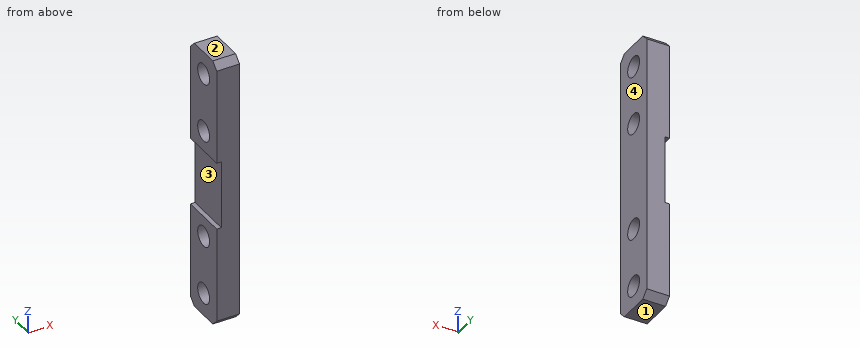
from build123d import *

# Parameters (mm, degrees)
SKETCH_1_W            = 120
SKETCH_1_H            = 20
EXTRUDE_1_DEPTH       = 10
HOLE_WIZARD_9_0_9_1_D = 9
HOLE_WIZARD_9_0_9_2_D = 9
SKETCH_6_W            = 30
SKETCH_6_H            = 20
CUT_EXTRUDE_1_DEPTH   = 2
CHAMFER_1_SIZE        = 3


with BuildPart() as part:
    # 草图1 → 凸台-拉伸1 (new body)
    with BuildSketch(Plane(origin=(0, 0, 0), x_dir=(0, 0, -1), z_dir=(1, 0, 0))):
        Rectangle(SKETCH_1_W, SKETCH_1_H)
    extrude(amount=EXTRUDE_1_DEPTH)

    # Ø9.0 (9) 直径孔1 (through all)
    with Locations(Plane(origin=(10, 0, 0), x_dir=(0, 0, -1), z_dir=(1, 0, 0))):
        with Locations((-24, 0), (24, 0)):
            Hole(HOLE_WIZARD_9_0_9_1_D / 2)

    # Ø9.0 (9) 直径孔2 (through all)
    with Locations(Plane.ZY):
        with Locations((-50, 0), (50, 0)):
            Hole(HOLE_WIZARD_9_0_9_2_D / 2)

    # 草图6 → 切除-拉伸1 (cut)
    with BuildSketch(Plane(origin=(0, 0, 0), x_dir=(0, 0, -1), z_dir=(1, 0, 0))):
        Rectangle(SKETCH_6_W, SKETCH_6_H)
    extrude(amount=CUT_EXTRUDE_1_DEPTH, mode=Mode.SUBTRACT)

    # 倒角1
    chamfer_1_edges = [part.edges().sort_by_distance(p)[0] for p in [
        (5, -10, -60),
        (5, -10, 60),
        (5, 10, 60),
        (5, 10, -60),
    ]]
    chamfer(chamfer_1_edges, length=CHAMFER_1_SIZE)


solid = part.part
Work out the finished part from the listing and answer in its coordinate system (mm). Face numbers are marked on the shaded views. Give positions to 0.01 mm unless a question says otherwise; leave off trailing zeros. Write each loop counter-clockwise with the first axis right and the second up, starting at its lowest first coordinate (ties: lowest second). Pieces come first, ordered by that corner, then holes.
Q1. For a pull along Z with two mould halves and no side action, classify the marked faces 1, 2, 3 and 4 as released by +Z, released by -Z, zero draft, split by the parting line, or undercut.
Answer:
face 1: released by -Z
face 2: released by +Z
face 3: undercut
face 4: zero draft
Q2. The part is cut by section D-D on z = -13. Give the vertices of the cut face in (x, y).
Answer:
outline: (2, -10) - (10, -10) - (10, 10) - (2, 10) - close
Q3. Straight lines are drawn through the part: L1, parallel to Y at x = 3, z = -50; L2, parallel to Z at x = 5, y = 2.75; L3, parallel to X at y = -7.25, z = 11.5. For each, find the intervals that lie inside material, in ascending order.
Answer:
L1: y = -10 to -4.5, 4.5 to 10
L2: z = -60 to -53.56, -46.44 to -27.56, -20.44 to 20.44, 27.56 to 46.44, 53.56 to 60
L3: x = 2 to 10
Q4. The part is cut by section B-B on y = 0. Give the vertices of the cut face in (x, z), and give its area (3 significant figures).
Answer:
outline: (0, -60) - (10, -60) - (10, -54.5) - (0, -54.5) - close; (0, -45.5) - (10, -45.5) - (10, -28.5) - (0, -28.5) - close; (0, -19.5) - (10, -19.5) - (10, 19.5) - (0, 19.5) - (0, 15) - (2, 15) - (2, -15) - (0, -15) - close; (0, 28.5) - (10, 28.5) - (10, 45.5) - (0, 45.5) - close; (0, 54.5) - (10, 54.5) - (10, 60) - (0, 60) - close
area: 780 mm2
Q5. The part is cut by section C-C on x = 7.25. Give the vertices of the cut face in (y, z).
Answer:
outline: (-10, -57) - (-7, -60) - (7, -60) - (10, -57) - (10, 57) - (7, 60) - (-7, 60) - (-10, 57) - close; hole circle Ø9 at (0, -50); hole circle Ø9 at (0, -24); hole circle Ø9 at (0, 24); hole circle Ø9 at (0, 50)
Q6. The part is cut by section A-A on z = -50. Give the vertices of the cut face in (x, y), and give its area (3 significant figures).
Answer:
outline: (0, -10) - (10, -10) - (10, -4.5) - (0, -4.5) - close; (0, 4.5) - (10, 4.5) - (10, 10) - (0, 10) - close
area: 110 mm2
